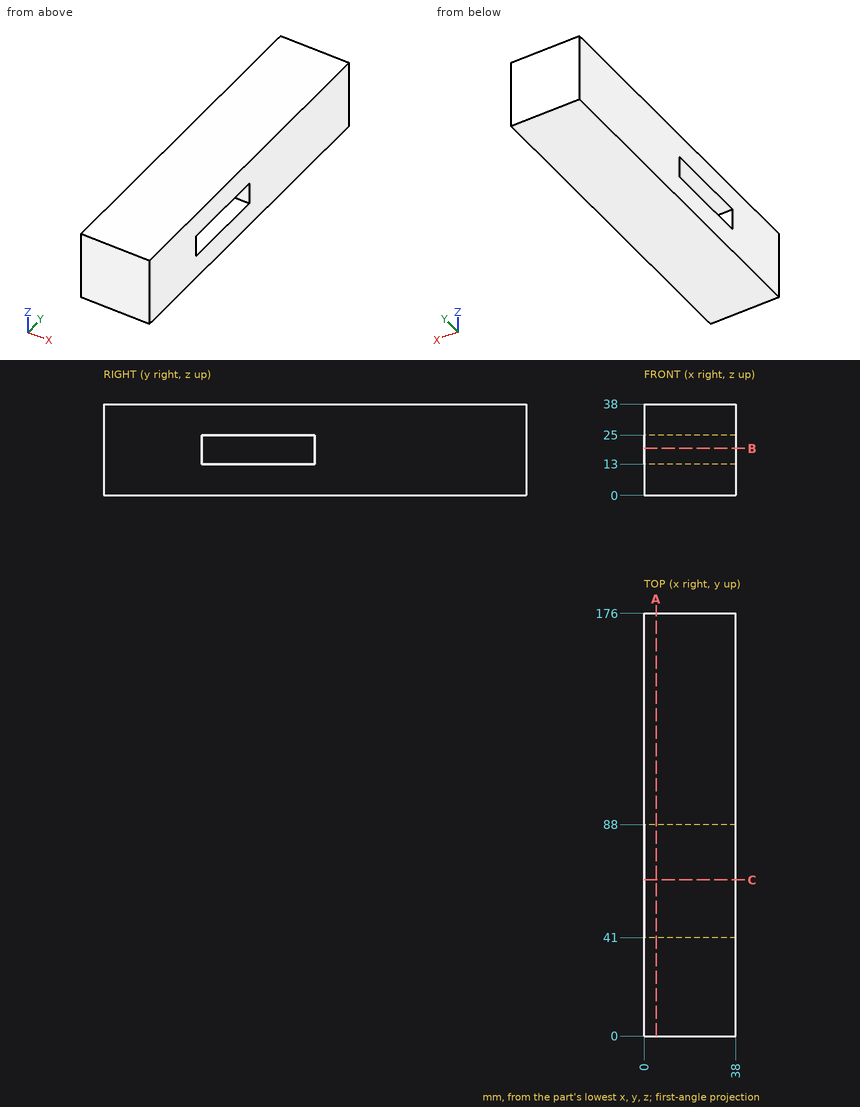
Verification items for this drawing (mm, ordinates from the low corner). Give positions to 0.01 mm unless a question says otherwise; leave off trailing zeros. Write each loop counter-clockwise with the first axis right and the second up, starting at its lowest first coordinate (ties: lowest second). Pieces come first, ordered by that corner, then holes. Notation, with made-up numbers: M -30,-13 L -7,-13 A20 cw -7,-7 Z; hole C -32,65.25 d1. An arc over 180 degrees is marked long. Use one line per item in the form item = value.
(1) Depth check by flat-ended pin: P1, Ø5, axis at x = 25, z = 31, coming from the -Y side. Enter the tip coordinate at first touch or a pass-through.
Answer block:
P1 = 0
(2) Material ranges on line 1 along Z through (x, y) = (32.5, 52.5); line 2 along Y through (x, z) = (21.5, 24.5), recorded low to high.
Answer block:
line_1 = 0 to 13, 25 to 38
line_2 = 0 to 41, 88 to 176
(3) Section check C-C on y = 65. Record the boundary of the cut face in (x, z), plus the area to 3 significant figures.
Answer block:
outline = M 0,0 L 38,0 L 38,13 L 0,13 Z; M 0,25 L 38,25 L 38,38 L 0,38 Z
area = 988 mm2
(4) Section check A-A on x = 5. Record the boundary of the cut face in (y, z), plus the area to 3 significant figures.
Answer block:
outline = M 0,0 L 176,0 L 176,38 L 0,38 Z; hole M 41,13 L 88,13 L 88,25 L 41,25 Z
area = 6,120 mm2
(5) Section check B-B on z = 19.5. Record the boundary of the cut face in (x, y), plus the area to 3 significant figures.
Answer block:
outline = M 0,0 L 38,0 L 38,41 L 0,41 Z; M 0,88 L 38,88 L 38,176 L 0,176 Z
area = 4,900 mm2
